```python
from build123d import *

# Parameters (mm, degrees)
BOSS_EXTRUDE1_DEPTH   = 30
M30_CLEARANCE_HOLE1_D = 35
M45_CLEARANCE_HOLE1_D = 50
FILLET1_R             = 10


with BuildPart() as part:
    # Sketch1 → Boss-Extrude1 (new body)
    with BuildSketch(Plane.XY.offset(30)):
        with BuildLine():
            Line((59.464274989, 8), (39.642849993, 155.333333333))
            ThreePointArc((39.642849993, 155.333333333), (0, 190), (-39.642849993, 155.333333333))
            Line((-39.642849993, 155.333333333), (-59.464274989, 8))
            ThreePointArc((-59.464274989, 8), (0, -60), (59.464274989, 8))
        make_face()
    extrude(amount=-BOSS_EXTRUDE1_DEPTH)

    # M30 Clearance Hole1 (through all)
    with Locations(Plane(origin=(0, 0, 0), x_dir=(-1, 0, 0), z_dir=(0, 0, -1))):
        with Locations((0, 150)):
            Hole(M30_CLEARANCE_HOLE1_D / 2)

    # M45 Clearance Hole1 (through all)
    with Locations(Plane(origin=(0, 0, 0), x_dir=(-1, 0, 0), z_dir=(0, 0, -1))):
        with Locations((0, 0)):
            Hole(M45_CLEARANCE_HOLE1_D / 2)

    # Fillet1
    fillet1_edges = [part.edges().sort_by_distance(p)[0] for p in [
        (0, 190, 0),
        (-49.553562491, 81.666666667, 0),
        (0, -60, 0),
        (-49.553562491, 81.666666667, 30),
        (0, 190, 30),
        (49.553562491, 81.666666667, 30),
        (0, -60, 30),
        (49.553562491, 81.666666667, 0),
    ]]
    fillet(fillet1_edges, radius=FILLET1_R)


solid = part.part
```
For this review, take the finished solid that the model builds, in its own axes (mm). Coordinates: 2 decimals unless noted, no trailing zeros. Order: outer loops, then holes, each group sorted by start corner. A loop starts at its lowest first (then second) coordinate and runs counter-clockwise, first axis right, second up. Notation, with made-up numbers: (88.25, -39) - (99.25, -39) arc R24 ccw to (99.25, -20) - close; hole circle Ø1 at (-15.75, 19.25). An arc over 180 degrees is marked (long way). Answer as a JSON object with one key per item and string values. Group by question number.
1. We need section B-B on z = 17.75. State the section outline as (x, y) points, then the cut area to 3 significant figures.
2. The part is to be moulded in two halves that separate along X. For faces 1 (the cylindrical face through (-2.28, 167.35, 15.21)), 2 (the cylindrical face through (-1.432, -59.983, 15.07)), 3 (the cylindrical face through (46.59, 82.32, 3.01)), say which applies: pulls with the +X half, pulls with the -X half, needs draft (parallel to the pull), parting line crosses it, or undercut.
3. For probe 1 along Y at (x, z) = (6.5, 27.25); probe 2 along X at (y, z) = (-3, 21.75); probe 3 along Y at (x, z) = (11, 12.25), list the stretches that pass through material, from the lowest coordinate up.
4. Clearance check with flat-ended pins moving along their axes: P1, Ø1.5, axis at y = -24, z = 14, coming from the +X side; P2, Ø4, axis at x = -35.5, z = 18, coming from the -Y side; P3, Ø3, axis at x = 25.5, z = 10, coming from the -Y side. State where each tip first meets the part, or that it passes through.
5. We need section A-A on x = 0. State the section outline as (y, z) points.
Final values:
{
 "1": {"outline": "(-59.46, 8) arc R60 ccw (long way) to (59.46, 8) - (39.64, 155.33) arc R40 ccw to (-39.64, 155.33) - close; hole circle Ø50 at (0, 0); hole circle Ø35 at (0, 150)", "area": "20,400 mm²"},
 "2": {"face 1": "undercut", "face 2": "parting line crosses it", "face 3": "pulls with the +X half"},
 "3": {"probe 1": "-56.51 to -24.14, 24.14 to 133.75, 166.25 to 186.31", "probe 2": "-59.77 to -24.82, 24.82 to 59.77", "probe 3": "-58.98 to -22.45, 22.45 to 136.39, 163.61 to 188.46"},
 "4": {"P1": "x = 55.31", "P2": "y = -49.78", "P3": "y = -54.99"},
 "5": {"outline": "(-60, 10) arc R10 ccw to (-50, 0) - (-25, 0) - (-25, 30) - (-50, 30) arc R10 ccw to (-60, 20) - close; (25, 0) - (132.5, 0) - (132.5, 30) - (25, 30) - close; (167.5, 0) - (180, 0) arc R10 ccw to (190, 10) - (190, 20) arc R10 ccw to (180, 30) - (167.5, 30) - close"}
}
